```python
from build123d import *

# Parameters (mm, degrees)
SKETCH_1_W                = 230
SKETCH_1_H                = 205
EXTRUDE_1_DEPTH           = 10
HOLE_WIZARD_1_D           = 5.5
HOLE_WIZARD_1_DEPTH       = 12.4
HOLE_WIZARD_1_CBORE_D     = 10
HOLE_WIZARD_1_CBORE_DEPTH = 5.7
HOLE_WIZARD_1_TIP         = 1.652366702
HOLE_WIZARD_2_D           = 5.5
HOLE_WIZARD_2_DEPTH       = 12.4
HOLE_WIZARD_2_CBORE_D     = 10
HOLE_WIZARD_2_CBORE_DEPTH = 5.7
HOLE_WIZARD_2_TIP         = 1.652366702
CHAMFER_1_SIZE            = 5
HOLE_WIZARD_3_D           = 6.6
HOLE_WIZARD_3_DEPTH       = 12.4
HOLE_WIZARD_3_CBORE_D     = 11
HOLE_WIZARD_3_CBORE_DEPTH = 6.8
HOLE_WIZARD_3_TIP         = 1.982840043


with BuildPart() as part:
    # 草图1 → 凸台-拉伸1 (new body)
    with BuildSketch(Plane(origin=(0, 0, 0), x_dir=(1, 0, 0), z_dir=(0, 1, 0))):
        Rectangle(SKETCH_1_W, SKETCH_1_H)
    extrude(amount=EXTRUDE_1_DEPTH)

    # 打孔尺寸(%根据)内六角圆柱头螺钉的类型1
    with Locations(Plane(origin=(0, 0, 0), x_dir=(-1, 0, 0), z_dir=(0, -1, 0))):
        with Locations((-95, -84.75), (-95, 85.25), (95, -84.75), (95, 85.25)):
            CounterBoreHole(HOLE_WIZARD_1_D / 2, HOLE_WIZARD_1_CBORE_D / 2, HOLE_WIZARD_1_CBORE_DEPTH, depth=HOLE_WIZARD_1_DEPTH)
            with Locations((0, 0, -(HOLE_WIZARD_1_DEPTH + HOLE_WIZARD_1_TIP / 2))):  # 118° drill point
                Cone(0, HOLE_WIZARD_1_D / 2, HOLE_WIZARD_1_TIP, mode=Mode.SUBTRACT)

    # 打孔尺寸(%根据)内六角圆柱头螺钉的类型2
    with Locations(Plane(origin=(0, 10, 0), x_dir=(1, 0, 0), z_dir=(0, 1, 0))):
        with Locations((-100, 0), (-70, 0), (-40, 0), (-20, 0), (-20, 40), (-20, -40), (20, -40), (40, 0), (20, 0), (70, 0), (100, 0), (20, 40)):
            CounterBoreHole(HOLE_WIZARD_2_D / 2, HOLE_WIZARD_2_CBORE_D / 2, HOLE_WIZARD_2_CBORE_DEPTH, depth=HOLE_WIZARD_2_DEPTH)
            with Locations((0, 0, -(HOLE_WIZARD_2_DEPTH + HOLE_WIZARD_2_TIP / 2))):  # 118° drill point
                Cone(0, HOLE_WIZARD_2_D / 2, HOLE_WIZARD_2_TIP, mode=Mode.SUBTRACT)

    # 倒角1
    chamfer_1_edges = [part.edges().sort_by_distance(p)[0] for p in [
        (115, 5, 102.5),
        (-115, 5, 102.5),
        (-115, 5, -102.5),
        (115, 5, -102.5),
    ]]
    chamfer(chamfer_1_edges, length=CHAMFER_1_SIZE)

    # 打孔尺寸(%根据)内六角圆柱头螺钉的类型3
    with Locations(Plane(origin=(0, 10, 0), x_dir=(1, 0, 0), z_dir=(0, 1, 0))):
        with Locations((0, 82.5), (0, 32.5), (0, -32.5), (0, -82.5)):
            CounterBoreHole(HOLE_WIZARD_3_D / 2, HOLE_WIZARD_3_CBORE_D / 2, HOLE_WIZARD_3_CBORE_DEPTH, depth=HOLE_WIZARD_3_DEPTH)
            with Locations((0, 0, -(HOLE_WIZARD_3_DEPTH + HOLE_WIZARD_3_TIP / 2))):  # 118° drill point
                Cone(0, HOLE_WIZARD_3_D / 2, HOLE_WIZARD_3_TIP, mode=Mode.SUBTRACT)


solid = part.part
```
Part model, mm, in its own coordinate system. A direction names the side the tool comes from. Round coordinates to 2 decimals unless told otherwise and drop trailing zeros. Loops run counter-clockwise (first coordinate to the right, second up) from the corner with the lowest first, then second, coordinate; pieces in that order, holes last. Notation, with made-up numbers: (-3, 0.5) -> (15, 0.5) arc R22 ccw to (15, 17.5) -> close; hole circle Ø2 at (29.25, 58). An arc over 180 degrees is marked (long way). Use one line per item in the form item = value. Start each with the question number.
Item 1: Band-saw the part on B-B (x = 40). List the corners of the cut face in (y, z), plus the area to 3 significant figures.
Item 2: Drill centre lines: line 1 along X through (y, z) = (1, -40); line 2 along X through (y, z) = (8.8, 84.75); line 3 along Z through (x, y) = (100, 7.15). Where is each one in solid material? Low to high.
Item 3: Band-saw the part on A-A (x = -20). List the corners of the cut face in (y, z).
Item 4: Band-saw the part on C-C (z = -32.5). List the corners of the cut face in (x, y), plus the area to 3 significant figures.
Item 5: Two-plate mould, pull along Z, no slides. Class faces 1 (the flat face through (112.5, 4.9, -100)), 2 (the cylindrical face through (72.747, 2.12, -0.121)), 3 (the flat face through (-2, 0, -1)): released by +Z, released by -Z, zero draft, split by the parting line, or undercut.
Item 6: Drop a flat-ended pin along its axis: pin 1 Ø6.5 at (x, z) = (100, 0) entering from +Y. Give the stop position or say it passes through.
Item 7: Tool access for faces 4 (the cylindrical face through (90.381, 2.81, 86.665)), 5 (the cylindrical face through (-97.253, 2.12, -0.121)), 6 (the cylindrical face through (-0.716, 6.648, -37.953)): list every direction of +Z, -Z, +X, -X, +Y, -Y with a clear straight run to the whole face (end or side of a thin tool).
Data:
q1.outline = (0, -102.5) -> (10, -102.5) -> (10, -5) -> (4.3, -5) -> (4.3, -2.75) -> (0, -2.75) -> close; (0, 2.75) -> (4.3, 2.75) -> (4.3, 5) -> (10, 5) -> (10, 102.5) -> (0, 102.5) -> close
q1.area = 1,970 mm^2
q2.line_1 = -115 to -22.75, -17.25 to 17.25, 22.75 to 115
q2.line_2 = -115 to -97.75, -92.25 to -5.02, 5.02 to 92.25, 97.75 to 115
q2.line_3 = -102.5 to -5, 5 to 102.5
q3.outline = (0, -102.5) -> (10, -102.5) -> (10, -45) -> (4.3, -45) -> (4.3, -42.75) -> (0, -42.75) -> close; (0, -37.25) -> (4.3, -37.25) -> (4.3, -35) -> (10, -35) -> (10, -5) -> (4.3, -5) -> (4.3, -2.75) -> (0, -2.75) -> close; (0, 2.75) -> (4.3, 2.75) -> (4.3, 5) -> (10, 5) -> (10, 35) -> (4.3, 35) -> (4.3, 37.25) -> (0, 37.25) -> close; (0, 42.75) -> (4.3, 42.75) -> (4.3, 45) -> (10, 45) -> (10, 102.5) -> (0, 102.5) -> close
q4.outline = (-115, 0) -> (-3.3, 0) -> (-3.3, 3.2) -> (-5.5, 3.2) -> (-5.5, 10) -> (-115, 10) -> close; (3.3, 0) -> (115, 0) -> (115, 10) -> (5.5, 10) -> (5.5, 3.2) -> (3.3, 3.2) -> close
q4.area = 2,200 mm^2
q5.face_1 = released by -Z
q5.face_2 = undercut
q5.face_3 = zero draft
q6.pin_1 = 4.3
q7.face_4 = -Y
q7.face_5 = +Y, -Y
q7.face_6 = +Y
